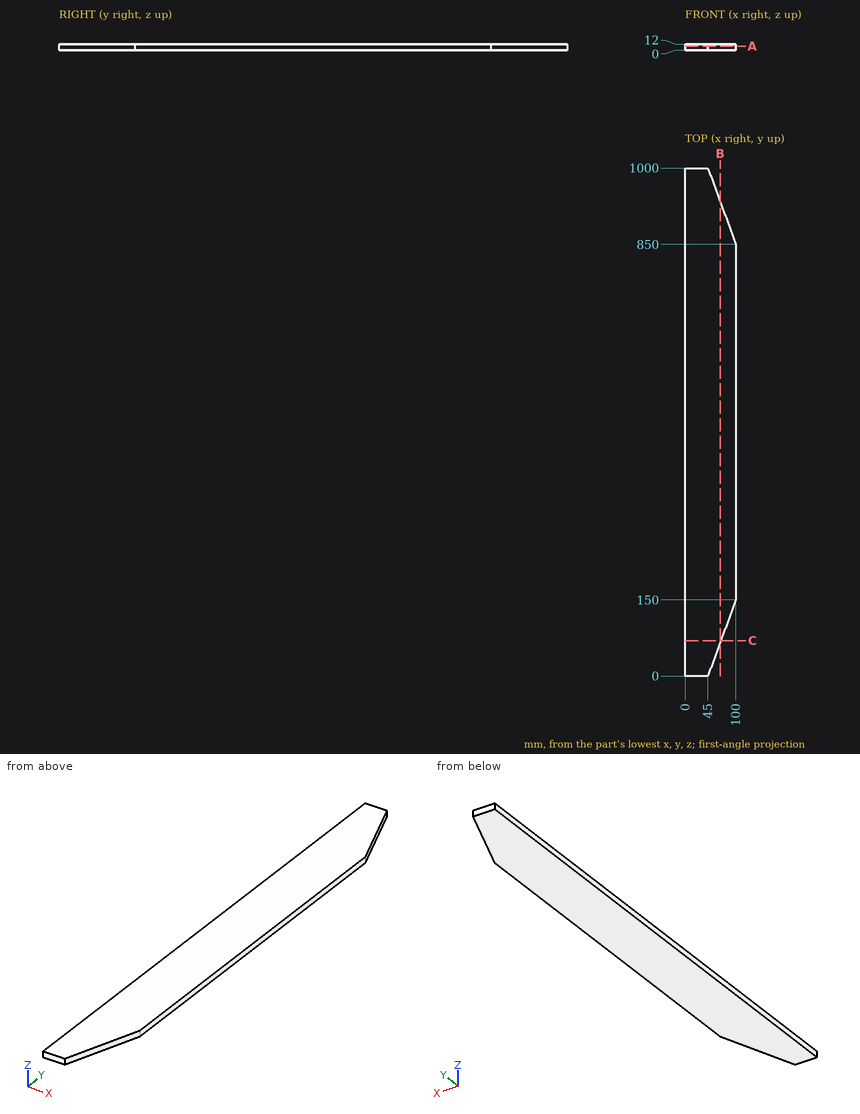
The drawing under review shows one solid part. Ordinate dimensions are in mm from its lowest x, y, z. Coordinates: 2 decimals unless noted, no trailing zeros. Write each loop counter-clockwise with the first axis right and the second up, starting at its lowest first coordinate (ties: lowest second). Pieces come first, ordered by that corner, then holes. Notation, with made-up numbers: M 70,8.5 L 128,8.5 A6 ccw 128,15.5 Z; hole C -21.75,34 d4. An arc over 180 degrees is marked long. Put each result on its own line as item: value.
1) Wall thickness on probe 1 along X at (y, z) = (132, 6); probe 2 along X at (y, z) = (49.5, 10.5): over which ranges is each line inside the solid? List them lowest first. Write a range as [from, to].
Computed:
probe 1: x = [0, 93.4]
probe 2: x = [0, 63.15]
2) Add section C-C on y = 69.5. Give the boundary of the cut face in (x, z).
Computed:
outline: M 0,0 L 70.48,0 L 70.48,12 L 0,12 Z
3) Add section B-B on x = 69. Give the boundary of the cut face in (y, z), then the cut area to 3 significant figures.
Computed:
outline: M 65.45,0 L 934.55,0 L 934.55,12 L 65.45,12 Z
area: 10,400 mm2
4) Add section A-A on z = 7.75. Give the boundary of the cut face in (x, y), then the cut area to 4 significant figures.
Computed:
outline: M 0,0 L 45,0 L 100,150 L 100,850 L 45,1000 L 0,1000 Z
area: 91,750 mm2
